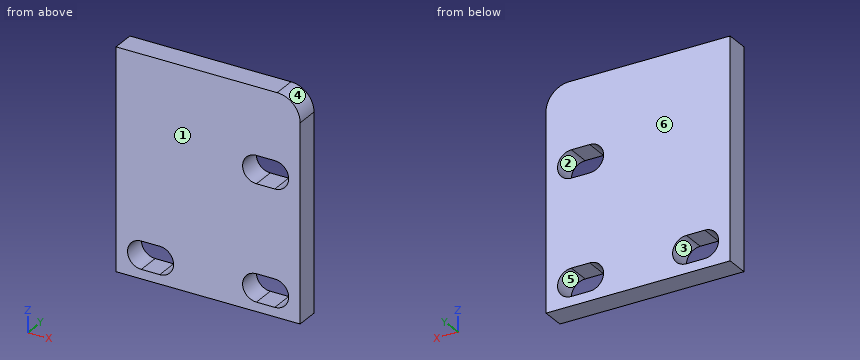
```python
from build123d import *

# Parameters (mm, degrees)
BOSS_EXTRUDE1_DEPTH = 10


with BuildPart() as part:
    # Sketch1 → Boss-Extrude1 (new body)
    with BuildSketch(Plane(origin=(0, 0, 0), x_dir=(1, 0, 0), z_dir=(0, 1, 0))):
        with BuildLine():
            Line((-40, -47.5), (30, -47.5))
            ThreePointArc((30, -47.5), (37.071067812, -44.571067812), (40, -37.5))
            Line((40, -37.5), (40, 47.5))
            Line((40, 47.5), (-40, 47.5))
            Line((-40, 47.5), (-40, -47.5))
        make_face()
        with BuildLine():
            Line((-29, 43.5), (-21, 43.5))
            ThreePointArc((-21, 43.5), (-15, 37.5), (-21, 31.5))
            Line((-21, 31.5), (-29, 31.5))
            ThreePointArc((-29, 31.5), (-35, 37.5), (-29, 43.5))
        make_face(mode=Mode.SUBTRACT)
        with BuildLine():
            Line((21, 31.5), (29, 31.5))
            ThreePointArc((29, 31.5), (35, 37.5), (29, 43.5))
            Line((29, 43.5), (21, 43.5))
            ThreePointArc((21, 43.5), (15, 37.5), (21, 31.5))
        make_face(mode=Mode.SUBTRACT)
        with BuildLine():
            Line((21, -18.5), (29, -18.5))
            ThreePointArc((29, -18.5), (35, -12.5), (29, -6.5))
            Line((29, -6.5), (21, -6.5))
            ThreePointArc((21, -6.5), (15, -12.5), (21, -18.5))
        make_face(mode=Mode.SUBTRACT)
    extrude(amount=BOSS_EXTRUDE1_DEPTH)


solid = part.part
```
Here's how the part is built. I have some questions about the finished solid (model axes, mm). Face numbers are marked on the shaded views. A direction names the side the tool comes from. Coordinates: 2 decimals unless noted, no trailing zeros. Loops run counter-clockwise (first coordinate to the right, second up) from the corner with the lowest first, then second, coordinate; pieces in that order, holes last. Notation, with made-up numbers: (85.25, 34.5) - (143.25, 34.5) arc R9 cw to (143.25, 51.5) - close; hole circle Ø3 at (14, -15.5). An arc over 180 degrees is marked (long way). Answer as CSV lines item,"result".
Q1. If we section it at B-B, the plane y = 2.75: Write out the boundary of the cut face in (x, z).
Response:
outline,"(-40, -47.5) - (40, -47.5) - (40, 37.5) arc R10 ccw to (30, 47.5) - (-40, 47.5) - close; hole (-29, -43.5) - (-21, -43.5) arc R6 ccw to (-21, -31.5) - (-29, -31.5) arc R6 ccw to start; hole (21, -43.5) - (29, -43.5) arc R6 ccw to (29, -31.5) - (21, -31.5) arc R6 ccw to start; hole (21, 6.5) - (29, 6.5) arc R6 ccw to (29, 18.5) - (21, 18.5) arc R6 ccw to start"
Q2. If we section it at C-C, the plane z = 12.5: Write out the boundary of the cut face in (x, y).
Response:
outline,"(-40, 0) - (15, 0) - (15, 10) - (-40, 10) - close; (35, 0) - (40, 0) - (40, 10) - (35, 10) - close"
Q3. If we section it at D-D, the plane x = -32: Write out the boundary of the cut face in (y, z).
Response:
outline,"(0, -47.5) - (10, -47.5) - (10, -42.7) - (0, -42.7) - close; (0, -32.3) - (10, -32.3) - (10, 47.5) - (0, 47.5) - close"
Q4. If I drill on L1, parallel to Z at x = 25.5, y = 3.5; L2, parallel to Z at x = 16.5, y = 2; L3, parallel to X at y = 1, z = 13.5, over which ranges is the centre line in solid material (lowest first)? Write a range as [from, to].
Response:
L1,"[-47.5, -43.5], [-31.5, 6.5], [18.5, 47.5]"
L2,"[-47.5, -41.47], [-33.53, 8.53], [16.47, 47.5]"
L3,"[-40, 15.08], [34.92, 40]"
Q5. If we section it at A-A, the plane z = -37.5: Write out the boundary of the cut face in (x, y), and give its area (3 significant figures).
Response:
outline,"(-40, 0) - (-35, 0) - (-35, 10) - (-40, 10) - close; (-15, 0) - (15, 0) - (15, 10) - (-15, 10) - close; (35, 0) - (40, 0) - (40, 10) - (35, 10) - close"
area,"400 mm2"
Q6. For the marked faces 5 and 6, which set-ups out of +Z, -Z, +X, -X, +Y, -Y let a thin tool reach every point of the face, with its end or its side?
Response:
face 5,"+Y, -Y"
face 6,"+Z, -Z, +X, -X, +Y"
Q7. We'd pull the mould along Z, two halves only. Please class the marked faces 1, 2, 3 and 4: pulls with the +Z half, pulls with the -Z half, needs draft (parallel to the pull), parting line crosses it, or undercut.
Response:
face 1,"needs draft"
face 2,"undercut"
face 3,"undercut"
face 4,"pulls with the +Z half"
